```python
from build123d import *

# Parameters (mm, degrees)
SKETCH1_W                                            = 104
SKETCH1_H                                            = 12
BOSS_EXTRUDE1_DEPTH                                  = 38
SKETCH2_W                                            = 5
SKETCH2_H                                            = 12
CUT_EXTRUDE1_DEPTH                                   = 112.373246339
SKETCH3_R                                            = 16
CUT_EXTRUDE2_DEPTH                                   = 112.373246339
SKETCH4_W                                            = 24
SKETCH4_H                                            = 12
BOSS_EXTRUDE2_DEPTH                                  = 10
SKETCH5_W                                            = 24
SKETCH5_H                                            = 12
BOSS_EXTRUDE3_DEPTH                                  = 10
CHAMFER1_SIZE                                        = 1
FILLET1_R                                            = 2
HOLE_SIZE_PER_SOCKET_HEAD_CAP_SCREW_TYPE_D           = 3.4
HOLE_SIZE_PER_SOCKET_HEAD_CAP_SCREW_TYPE_CBORE_D     = 5.5
HOLE_SIZE_PER_SOCKET_HEAD_CAP_SCREW_TYPE_CBORE_DEPTH = 4
SKETCH8_R                                            = 2.5
CUT_EXTRUDE3_DEPTH                                   = 2.1
HOLE_SIZE_PER_SOCKET_HEAD_CAP_SCREW_2_D              = 5.5
HOLE_SIZE_PER_SOCKET_HEAD_CAP_SCREW_2_CBORE_D        = 10
HOLE_SIZE_PER_SOCKET_HEAD_CAP_SCREW_2_CBORE_DEPTH    = 6
SKETCH11_R                                           = 4.5
CUT_EXTRUDE4_DEPTH                                   = 2.1
M4_TAPPED_HOLE1_D                                    = 3.3
M4_TAPPED_HOLE1_DEPTH                                = 11.5
M4_TAPPED_HOLE1_TIP                                  = 0.991420021


with BuildPart() as part:
    # Sketch1 → Boss-Extrude1 (new body)
    with BuildSketch(Plane.XY):
        with Locations((52, 6)):
            Rectangle(SKETCH1_W, SKETCH1_H)
    extrude(amount=BOSS_EXTRUDE1_DEPTH)

    # Sketch2 → Cut-Extrude1 (cut, through all)
    with BuildSketch(Plane(origin=(0, 12, 0), x_dir=(1, 0, 0), z_dir=(0, 1, 0))):
        with Locations((2.5, -19)):
            Rectangle(SKETCH2_W, SKETCH2_H)
    extrude(amount=-CUT_EXTRUDE1_DEPTH, mode=Mode.SUBTRACT)

    # Sketch3 → Cut-Extrude2 (cut, through all)
    with BuildSketch(Plane(origin=(0, 12, 0), x_dir=(1, 0, 0), z_dir=(0, 1, 0))):
        with Locations((104, -19)):
            Circle(SKETCH3_R)
    extrude(amount=-CUT_EXTRUDE2_DEPTH, mode=Mode.SUBTRACT)

    # Sketch4 → Boss-Extrude2 (add)
    with BuildSketch(Plane(origin=(0, 0, 0), x_dir=(-1, 0, 0), z_dir=(0, 0, -1))):
        with Locations((-92, 6)):
            Rectangle(SKETCH4_W, SKETCH4_H)
    extrude(amount=BOSS_EXTRUDE2_DEPTH)

    # Sketch5 → Boss-Extrude3 (add)
    with BuildSketch(Plane.XY.offset(38)):
        with Locations((92, 6)):
            Rectangle(SKETCH5_W, SKETCH5_H)
    extrude(amount=BOSS_EXTRUDE3_DEPTH)

    # Chamfer1
    chamfer1_edges = [part.edges().sort_by_distance(p)[0] for p in [
        (0, 6, 0),
        (0, 6, 38),
        (104, 6, 48),
        (80, 6, 48),
        (104, 6, -10),
        (80, 6, -10),
    ]]
    chamfer(chamfer1_edges, length=CHAMFER1_SIZE)

    # Fillet1
    fillet1_edges = [part.edges().sort_by_distance(p)[0] for p in [
        (80, 6, 38),
        (80, 6, 0),
    ]]
    fillet(fillet1_edges, radius=FILLET1_R)

    # Hole size per socket head cap screw type (through all)
    with Locations(Plane(origin=(0, 0, 0), x_dir=(-1, 0, 0), z_dir=(0, -1, 0))):
        with Locations((-3, -35), (-21, -3), (-3, -3), (-21, -35)):
            CounterBoreHole(HOLE_SIZE_PER_SOCKET_HEAD_CAP_SCREW_TYPE_D / 2, HOLE_SIZE_PER_SOCKET_HEAD_CAP_SCREW_TYPE_CBORE_D / 2, HOLE_SIZE_PER_SOCKET_HEAD_CAP_SCREW_TYPE_CBORE_DEPTH)

    # Sketch8 → Cut-Extrude3 (cut)
    with BuildSketch(Plane(origin=(0, 12, 0), x_dir=(1, 0, 0), z_dir=(0, 1, 0))):
        with Locations(Location((3, -35, 0), (0, 0, 270))):
            Circle(SKETCH8_R)
        with Locations(Location((21, -3, 0), (0, 0, 270))):
            Circle(SKETCH8_R)
    extrude(amount=-CUT_EXTRUDE3_DEPTH, mode=Mode.SUBTRACT)

    # Hole size per socket head cap screw  2 (through all)
    with Locations(Plane(origin=(0, 12, 0), x_dir=(1, 0, 0), z_dir=(0, 1, 0))):
        with Locations((28.5, -10), (28.5, -30), (58.5, -10), (58.5, -30)):
            CounterBoreHole(HOLE_SIZE_PER_SOCKET_HEAD_CAP_SCREW_2_D / 2, HOLE_SIZE_PER_SOCKET_HEAD_CAP_SCREW_2_CBORE_D / 2, HOLE_SIZE_PER_SOCKET_HEAD_CAP_SCREW_2_CBORE_DEPTH)

    # Sketch11 → Cut-Extrude4 (cut)
    with BuildSketch(Plane.XZ):
        with Locations(Location((28.5, 30, 0), (0, 0, 270))):
            Circle(SKETCH11_R)
        with Locations(Location((58.5, 10, 0), (0, 0, 270))):
            Circle(SKETCH11_R)
    extrude(amount=-CUT_EXTRUDE4_DEPTH, mode=Mode.SUBTRACT)

    # M4 Tapped Hole1
    with Locations(Plane(origin=(104, 0, 0), x_dir=(0, 0, -1), z_dir=(1, 0, 0))):
        with Locations((3, 6), (-41, 6)):
            Hole(M4_TAPPED_HOLE1_D / 2, depth=M4_TAPPED_HOLE1_DEPTH)
            with Locations((0, 0, -(M4_TAPPED_HOLE1_DEPTH + M4_TAPPED_HOLE1_TIP / 2))):  # 118° drill point
                Cone(0, M4_TAPPED_HOLE1_D / 2, M4_TAPPED_HOLE1_TIP, mode=Mode.SUBTRACT)


solid = part.part
```
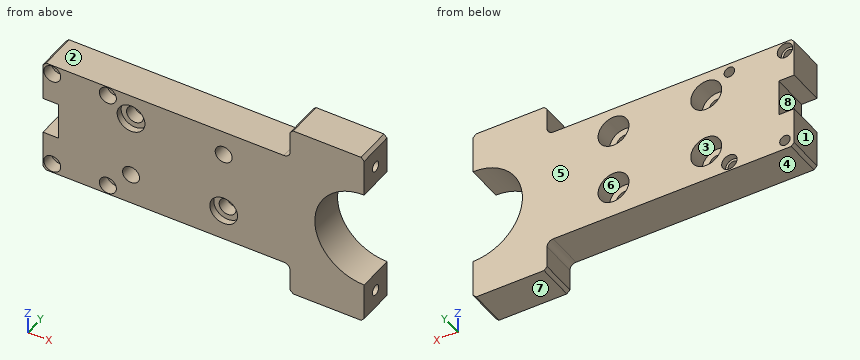
Input: part model. Units: mm. Frame: model coordinates. Face numbers are marked on the shaded views. A direction names the side the tool comes from. Give positions to 0.01 mm unless a question says otherwise; leave off trailing zeros. Order: outer loops, then holes, each group sorted by start corner. A loop starts at its lowest first (then second) coordinate and runs counter-clockwise, first axis right, second up.
1. Section A-A on x = 3. Return the cut outline in (y, z).
Derived:
outline: (0, 0) - (12, 0) - (12, 1.3) - (4, 1.3) - (4, 0.25) - (0, 0.25) - close; (0, 5.75) - (4, 5.75) - (4, 4.7) - (12, 4.7) - (12, 13) - (0, 13) - close; (0, 25) - (12, 25) - (12, 32.5) - (9.9, 32.5) - (9.9, 33.3) - (4, 33.3) - (4, 32.25) - (0, 32.25) - close; (0, 37.75) - (4, 37.75) - (4, 36.7) - (9.9, 36.7) - (9.9, 37.5) - (12, 37.5) - (12, 38) - (0, 38) - close
2. Reachability of the marked faces 4, 5, 6, 7 and 8 from +Z, -Z, +X, -X, +Y, -Y: full face, straight path, thin tool, end or side. Return the list, or none.
Derived:
face 4: -Z, -X, +Y, -Y
face 5: +Z, -Z, +X, -X, +Y
face 6: +Y
face 7: -Z, +X, -X, +Y, -Y
face 8: -X, +Y, -Y
3. Section C-C on z = 10. Return the cut outline in (x, y), and give its area (3 significant figures).
Derived:
outline: (0, 0) - (25.75, 0) - (25.75, 6) - (23.5, 6) - (23.5, 12) - (0, 12) - close; (31.25, 0) - (54, 0) - (54, 2.1) - (55.75, 2.1) - (55.75, 6) - (53.5, 6) - (53.5, 12) - (33.5, 12) - (33.5, 6) - (31.25, 6) - close; (61.25, 2.1) - (63, 2.1) - (63, 0) - (90.77, 0) - (90.77, 12) - (63.5, 12) - (63.5, 6) - (61.25, 6) - close
area: 896 mm2
4. Section D-D on z = 19. Return the cut outline in (x, y).
Derived:
outline: (5, 0) - (88, 0) - (88, 12) - (5, 12) - close
5. Section B-B on x = 58.5. Return the cut outline in (y, z).
Derived:
outline: (0, 0) - (12, 0) - (12, 5) - (6, 5) - (6, 7.25) - (2.1, 7.25) - (2.1, 5.5) - (0, 5.5) - close; (0, 14.5) - (2.1, 14.5) - (2.1, 12.75) - (6, 12.75) - (6, 15) - (12, 15) - (12, 25) - (6, 25) - (6, 27.25) - (0, 27.25) - close; (0, 32.75) - (6, 32.75) - (6, 35) - (12, 35) - (12, 38) - (0, 38) - close
6. Pin query (flat end, axial travel): pin 1 (8 mm diameter, centred on x = 3, z = 35, fed in from -Y); pin 2 (2 mm diameter, centred on y = 4.5, z = 32, fed in from +X); pin 3 (4.5 mm diameter, centred on x = 28.5, z = 30, fed in from +Y); pin 4 (1 mm diameter, centred on x = 19, y = 2, fed in from -Z). Return the tip coordinate at first contact, or that it passes through.
Derived:
pin 1: stops at y = 0
pin 2: stops at x = 96.25
pin 3: passes through
pin 4: stops at z = 0
7. Material intervals for L1, parallel to Z at x = 21, y = 6; L2, parallel to Z at x = 21, y = 2.15; L3, parallel to Z at x = 3, y = 8.75, sorted ascending.
Derived:
L1: z = 0 to 1.3, 4.7 to 33.3, 36.7 to 38
L2: z = 0 to 0.25, 5.75 to 32.25, 37.75 to 38
L3: z = 0 to 1.3, 4.7 to 13, 25 to 33.3, 36.7 to 38
8. Mould query, pull axis X, two halves, no side actions, for the marked faces 1, 2 and 3. Classes: released by +X, released by -X, zero draft, split by the parting line, or undercut.
Derived:
face 1: released by -X
face 2: zero draft
face 3: undercut
